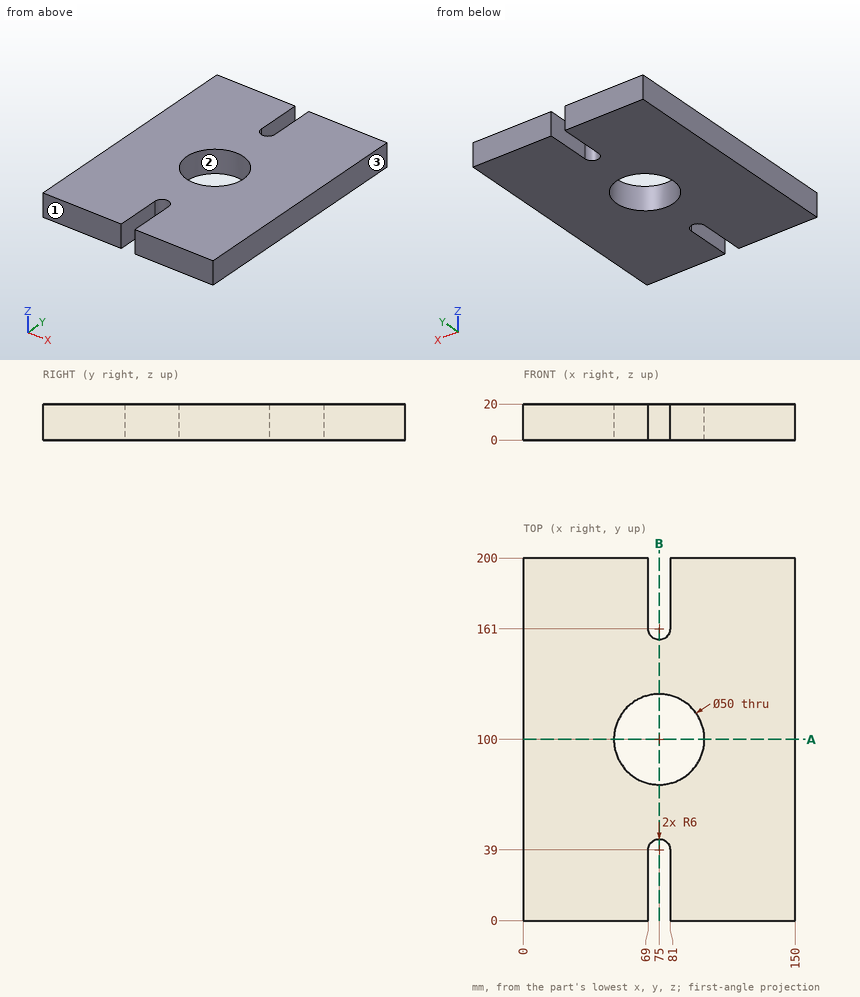
Geometry check sheet. Reference: drawing and pictorial views, mm from the part's lowest x, y, z. Round coordinates to 2 decimals unless told otherwise and drop trailing zeros. Order: outer loops, then holes, each group sorted by start corner. A loop starts at its lowest first (then second) coordinate and runs counter-clockwise, first axis right, second up. Notation, with made-up numbers: M 20,23.5 L 27,23.5 A19 cw 27,55.5 Z; hole C 68.25,54.5 d2. An arc over 180 degrees is marked long. Write item = value, one per line.
Q1. Scan lines: line 1 (Y direction, x = 75, z = 9); line 2 (X direction, y = 187.5, z = 16.25); line 3 (Y direction, x = 86, z = 15.75). Record each from-to range of solid material in increasing order.
Answer block:
line_1 = 45 to 75, 125 to 155
line_2 = 0 to 69, 81 to 150
line_3 = 0 to 77.55, 122.45 to 200
Q2. Release check for a two-part mould opening along X. For the marked faces 1, 2 and 3 record: released by +X, released by -X, zero draft, split by the parting line, or undercut.
Answer block:
face_1 = zero draft
face_2 = undercut
face_3 = released by +X
Q3. Section check B-B (x = 75). Enter the section's corners in (y, z), plus the area to 3 significant figures.
Answer block:
outline = M 45,0 L 75,0 L 75,20 L 45,20 Z; M 125,0 L 155,0 L 155,20 L 125,20 Z
area = 1,200 mm^2
Q4. Section check A-A (y = 100). Enter the section's corners in (x, z), plus the area to 3 significant figures.
Answer block:
outline = M 0,0 L 50,0 L 50,20 L 0,20 Z; M 100,0 L 150,0 L 150,20 L 100,20 Z
area = 2,000 mm^2
